Answer from the drawing. Dimensions are ordinates in mm from the lowest x, y and z of the part. Give positions to 0.01 mm unless a question says otherwise; leave off trailing zeros. Write each loop counter-clockwise with the first axis right and the second up, starting at its lowest first coordinate (ties: lowest second). Pieces come first, ordered by that corner, then holes. Notation, with made-up numbers: (7, -9) - (56, -9) arc R20 cw to (56, 16) - close; hole circle Ø5 at (-24.75, 88). An arc over 180 degrees is marked (long way). Answer as a JSON object with one key per item and string values. Group by question number.
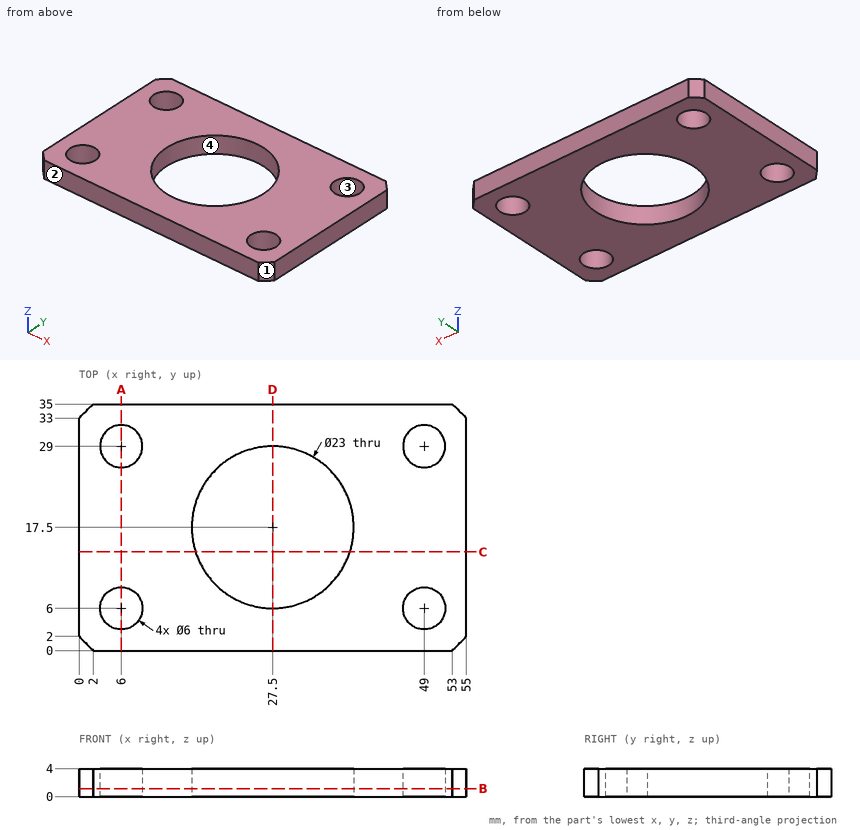
1) Find the intervals of material crossed by line 1 (Y direction, x = 49, z = 1.95); line 2 (Y direction, x = 50, z = 3.8); line 3 (X direction, y = 31, z = 2.6), in increasing order. Write a range as [from, to].
2) Find section C-C, the plane y = 14. Write down the section's boundary in (x, z), and give its area (3 significant figures).
3) Find section A-A, the plane x = 6. Write down the section's boundary in (y, z), and give its area (3 significant figures).
4) Find section D-D, the plane x = 27.5. Write down the section's boundary in (y, z).
5) Find section B-B, the plane z = 1.15. Write down the section's boundary in (x, y).
6) For a pull along X with two mould halves and no side action, classify the marked faces 1, 2, 3 and 4 as released by +X, released by -X, zero draft, split by the parting line, or undercut.
Values follow:
{
 "1": {"line 1": "y = [0, 3], [9, 26], [32, 35]", "line 2": "y = [0, 3.17], [8.83, 26.17], [31.83, 35]", "line 3": "x = [0, 3.76], [8.24, 46.76], [51.24, 55]"},
 "2": {"outline": "(0, 0) - (16.55, 0) - (16.55, 4) - (0, 4) - close; (38.45, 0) - (55, 0) - (55, 4) - (38.45, 4) - close", "area": "132 mm2"},
 "3": {"outline": "(0, 0) - (3, 0) - (3, 4) - (0, 4) - close; (9, 0) - (26, 0) - (26, 4) - (9, 4) - close; (32, 0) - (35, 0) - (35, 4) - (32, 4) - close", "area": "92.0 mm2"},
 "4": {"outline": "(0, 0) - (6, 0) - (6, 4) - (0, 4) - close; (29, 0) - (35, 0) - (35, 4) - (29, 4) - close"},
 "5": {"outline": "(0, 2) - (2, 0) - (53, 0) - (55, 2) - (55, 33) - (53, 35) - (2, 35) - (0, 33) - close; hole circle Ø6 at (6, 6); hole circle Ø6 at (6, 29); hole circle Ø23 at (27.5, 17.5); hole circle Ø6 at (49, 6); hole circle Ø6 at (49, 29)"},
 "6": {"face 1": "released by +X", "face 2": "zero draft", "face 3": "undercut", "face 4": "undercut"}
}
